Could you check a few things on this model? Use its own coordinates, in mm. Face numbers are marked on the shaded views. A direction names the side the tool comes from. Give positions to 0.01 mm unless a question says otherwise; leave off trailing zeros. Write each loop counter-clockwise with the first axis right and the second up, starting at its lowest first coordinate (ties: lowest second). Pieces come first, ordered by that corner, then holes. Notation, with made-up numbers: (59.25, 82) -> (118.25, 82) arc R9 cw to (118.25, 88) -> close; hole circle Ø11 at (-39.5, -27). An arc over 180 degrees is marked (long way). Write item = value, one per line. Start each with the question number.
```python
from build123d import *

# Parameters (mm, degrees)
SKETCH_1_W          = 9
SKETCH_1_H          = 40
EXTRUDE_1_DEPTH     = 6.3
SKETCH_2_W          = 9
SKETCH_2_H          = 24.3
EXTRUDE_2_DEPTH     = 5
CUT_EXTRUDE_1_DEPTH = 30.653667564
SKETCH_4_R          = 2.5
CUT_EXTRUDE_2_DEPTH = 44.062048256
FILLET_1_R          = 1
CHAMFER_2_SIZE      = 0.5


with BuildPart() as part:
    # 草图1 → 凸台-拉伸1 (new body)
    with BuildSketch(Plane.XY):
        Rectangle(SKETCH_1_W, SKETCH_1_H)
    extrude(amount=EXTRUDE_1_DEPTH)

    # 草图2 → 凸台-拉伸2 (add)
    with BuildSketch(Plane.XZ.offset(20)):
        with Locations((0, 3.15)):
            Rectangle(SKETCH_2_W, SKETCH_2_H)
    extrude(amount=EXTRUDE_2_DEPTH)

    # 草图3 → 切除-拉伸1 (cut, through all)
    with BuildSketch(Plane(origin=(0, 0, 0), x_dir=(-1, 0, 0), z_dir=(0, 0, -1))):
        Polygon((-2.5, 20), (4.5, 20), (4.5, 7.875644347), align=None)
    extrude(amount=-CUT_EXTRUDE_1_DEPTH, mode=Mode.SUBTRACT)

    # 草图4 → 切除-拉伸2 (cut, through all)
    with BuildSketch(Plane(origin=(0, -20, 0), x_dir=(1, 0, 0), z_dir=(0, 1, 0))):
        with Locations(Location((0, 4.5, 0), (0, 0, 270))):
            Circle(SKETCH_4_R)
        with Locations(Location((0, -10.8, 0), (0, 0, 270))):
            Circle(SKETCH_4_R)
    extrude(amount=-CUT_EXTRUDE_2_DEPTH, mode=Mode.SUBTRACT)

    # 圆角1
    fillet_1_edges = [part.edges().sort_by_distance(p)[0] for p in [
        (2.5, 20, 3.15),
    ]]
    fillet(fillet_1_edges, radius=FILLET_1_R)

    # 倒角2
    chamfer_2_edges = [part.edges().sort_by_distance(p)[0] for p in [
        (-4.5, -22.5, 15.3),
        (-4.5, -22.5, -9),
        (4.5, -22.5, -9),
        (4.5, -22.5, 15.3),
        (4.5, 20, 3.15),
    ]]
    chamfer(chamfer_2_edges, length=CHAMFER_2_SIZE)


solid = part.part
```
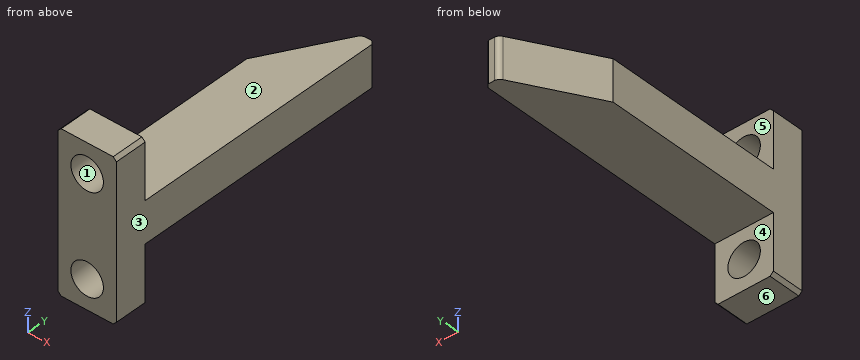
(1) Imagine slicing it at C-C (z = 2.25). Please give me the cut outline in (x, y), then the cut area to 3 significant figures.
(2) I'm going to push flat-ended pins straight in: pin 1 (4.5 mm diameter, centred on x = 0.5, z = 9, fed in from +Y); pin 2 (2 mm diameter, centred on x = -2, y = -18, fed in from +Z); pin 3 (6 mm diameter, centred on y = 11, z = 8.5, fed in from +X); pin 4 (4 mm diameter, centred on x = -2, y = 0, fed in from -Z). Where does each tip first touch, or does it pass through?
(3) Imagine slicing it at B-B (x = 3.5). Please give me the cut outline in (y, z).
(4) If I drill on line 1 along X through (y, z) = (-23.65, 10.8); line 2 along Z through (x, y) = (-0.5, 8); line 3 along Y through (x, z) = (-2.5, -3), over which ranges is the centre line in solid material (lowest first)? Write a range as from..to.
(5) On a 3-axis mill with a long thin cutter (end or side, diameter ignored), from which of +Z, -Z, +X, -X, +Y, -Y can I reach the whole of each face in a straight line? I mean the marked faces 4, 5 and 6. Say none if no direction works.
(6) We'd pull the mould along X, two halves only. Please class the marked faces 1, 2 and 3: released by +X, released by -X, zero draft, split by the parting line, or undercut.
(7) Imagine slicing it at A-A (z = -4.5). Please give me the cut outline in (x, y), then the cut area to 3 significant figures.
(8) Imagine slicing it at D-D (x = -1.75). Please give me the cut outline in (y, z).
Answers below:
q1.outline = (-4.5, -25) -> (4.5, -25) -> (4.5, 19.5) -> (4, 20) -> (3.08, 20) arc R1 ccw to (2.21, 19.5) -> (-4.5, 7.88) -> close
q1.area = 362 mm^2
q2.pin_1 = -20
q2.pin_2 = 6.3
q2.pin_3 = 4.5
q2.pin_4 = 0
q3.outline = (-25, -9) -> (-20, -9) -> (-20, 0) -> (20, 0) -> (20, 6.3) -> (-20, 6.3) -> (-20, 15.3) -> (-25, 15.3) -> close
q4.line_1 = -4.5..-2.5, 2.5..4.5
q4.line_2 = 0..6.3
q4.line_3 = -25..-20
q5.face_4 = -Z, +X, -X, +Y
q5.face_5 = +Z, +X, -X, +Y
q5.face_6 = -Z, +X, -X, +Y, -Y
q6.face_1 = undercut
q6.face_2 = zero draft
q6.face_3 = released by +X
q7.outline = (-4.5, -25) -> (-2.5, -25) -> (-2.5, -20) -> (-4.5, -20) -> close; (2.5, -25) -> (4.5, -25) -> (4.5, -20) -> (2.5, -20) -> close
q7.area = 20.0 mm^2
q8.outline = (-25, -9) -> (-20, -9) -> (-20, -6.29) -> (-25, -6.29) -> close; (-25, -2.71) -> (-20, -2.71) -> (-20, 0) -> (12.64, 0) -> (12.64, 6.3) -> (-20, 6.3) -> (-20, 9.01) -> (-25, 9.01) -> close; (-25, 12.59) -> (-20, 12.59) -> (-20, 15.3) -> (-25, 15.3) -> close
